Part model, mm, in its own coordinate system. A direction names the side the tool comes from. Round coordinates to 2 decimals unless told otherwise and drop trailing zeros. Answer as a JSON object with one key per item and string values.
```python
from build123d import *

# Parameters (mm, degrees)
SKETCH_1_W          = 180
SKETCH_1_H          = 30
EXTRUDE_1_DEPTH     = 20
SKETCH_2_R          = 2
CUT_EXTRUDE_1_DEPTH = 2


with BuildPart() as part:
    # 草图1 → 凸台-拉伸1 (new body)
    with BuildSketch(Plane.XY):
        Rectangle(SKETCH_1_W, SKETCH_1_H)
    extrude(amount=EXTRUDE_1_DEPTH)

    # 草图2 → 切除-拉伸1 (cut)
    with BuildSketch(Plane.XY.offset(20)):
        with Locations((-10, 0)):
            Circle(SKETCH_2_R)
        with Locations((10, 0)):
            Circle(SKETCH_2_R)
    extrude(amount=-CUT_EXTRUDE_1_DEPTH, mode=Mode.SUBTRACT)


solid = part.part
```
Item 1: Tool access for faces 1 (the flat face through (90, 0, 10)), 2 (the flat face through (-10, 0, 18)): list every direction of +Z, -Z, +X, -X, +Y, -Y with a clear straight run to the whole face (end or side of a thin tool).
Taken from the geometry:
{"face 1": "+Z, -Z, +X, +Y, -Y", "face 2": "+Z"}
Item 2: Drop a flat-ended pin along its axis: P1, Ø2, axis at x = 9.5, y = 0.5, coming from the +Z side. Give the stop position or say it passes through.
Taken from the geometry:
{"P1": "z = 18"}
Item 3: Probe L1, parallel to Y at x = 10, z = 19. List the from-to ranges inside material, lowest first. Write a range as from..to.
Taken from the geometry:
{"L1": "-15..-2, 2..15"}
Item 4: Two-plate mould, pull along Y, no slides. Class faces 3 (the flat face through (10, 0, 18)), 4 (the flat face through (-1, 15, 10)), 5 (the flat face through (-1, 0, 20)): pulls with the +Y half, pulls with the -Y half, needs draft (parallel to the pull), parting line crosses it, or undercut.
Taken from the geometry:
{"face 3": "undercut", "face 4": "pulls with the +Y half", "face 5": "needs draft"}
